from build123d import *

# Parameters (mm, degrees)
SKETCH_2_R              = 24
CUT_EXTRUDE_1_DEPTH     = 203.193286239
HOLE_WIZARD_M8_1_D      = 9
SKETCH_7_W              = 10
SKETCH_7_H              = 5
HOLE_WIZARD_M10_1_D     = 8.5
HOLE_WIZARD_M10_1_DEPTH = 24.5
HOLE_WIZARD_M10_1_TIP   = 2.553657631


with BuildPart() as part:
    # 草图1 → 旋转1 (revolve)
    with BuildSketch(Plane.XY, mode=Mode.PRIVATE) as revolve_1_sk:
        Polygon((0, 0), (87.5, 0), (87.5, 5), (111.25, 5), (111.25, 68), (80, 68), (80, 101), (42.5, 101), (42.5, 113), (27.5, 113), (27.5, 127), (0, 127), align=None)
    revolve(revolve_1_sk.sketch.rotate(Axis((0, 0, 0), (0, 1, 0)), 90), axis=Axis((0, 0, 0), (0, 1, 0)))

    # 草图2 → 切除-拉伸1 (cut, through all)
    with BuildSketch(Plane(origin=(0, 127, 0), x_dir=(1, 0, 0), z_dir=(0, 1, 0))):
        with Locations(Location((0, 0, 0), (0, 0, 270))):
            Circle(SKETCH_2_R)
    extrude(amount=-CUT_EXTRUDE_1_DEPTH, mode=Mode.SUBTRACT)

    # M8 间隙孔1 (through all)
    with Locations(Plane(origin=(0, 68, 0), x_dir=(1, 0, 0), z_dir=(0, 1, 0))):
        with Locations((0, 104), (73.539105243, 73.539105243), (104, 0), (73.539105243, -73.539105243), (0, -104), (-73.539105243, -73.539105243), (-104, 0), (-73.539105243, 73.539105243)):
            Hole(HOLE_WIZARD_M8_1_D / 2)

    # 草图7 → 切除-旋转1 (revolve, cut)
    with BuildSketch(Plane.XY, mode=Mode.PRIVATE) as cut_revolve_1_sk:
        with Locations((75, 91.5)):
            Rectangle(SKETCH_7_W, SKETCH_7_H)
    revolve(cut_revolve_1_sk.sketch.rotate(Axis((0, 0, 0), (0, 1, 0)), 90), axis=Axis((0, 0, 0), (0, 1, 0)), mode=Mode.SUBTRACT)

    # M10 螺纹孔1
    with Locations(Plane(origin=(0, 0, 0), x_dir=(-1, 0, 0), z_dir=(0, -1, 0))):
        with Locations((0, 67), (47.376154339, 47.376154339), (67, 0), (47.376154339, -47.376154339), (0, -67), (-47.376154339, -47.376154339), (-67, 0), (-47.376154339, 47.376154339)):
            Hole(HOLE_WIZARD_M10_1_D / 2, depth=HOLE_WIZARD_M10_1_DEPTH)
            with Locations((0, 0, -(HOLE_WIZARD_M10_1_DEPTH + HOLE_WIZARD_M10_1_TIP / 2))):  # 118° drill point
                Cone(0, HOLE_WIZARD_M10_1_D / 2, HOLE_WIZARD_M10_1_TIP, mode=Mode.SUBTRACT)


solid = part.part
Part model, mm, in its own coordinate system. A direction names the side the tool comes from. Round coordinates to 2 decimals unless told otherwise and drop trailing zeros. Order: outer loops, then holes, each group sorted by start corner. A loop starts at its lowest first (then second) coordinate and runs counter-clockwise, first axis right, second up. Notation, with made-up numbers: (-38.75, 51.5) -> (-14.75, 51.5) arc R20 ccw to (-14.75, 88.5) -> close; hole circle Ø7 at (38, 77). An arc over 180 degrees is marked (long way). Put each result on its own line as item: value.
Q1. Tool access for faces 4 (the face through (108.496, 36.059, -0.198)), 5 (the face through (71, 89, 0)), 6 (the face through (74, 68, -32)), 7 (the face through (-45.42, 12.42, 51.15)): list every direction of +Z, -Z, +X, -X, +Y, -Y with a clear straight run to the whole face (end or side of a thin tool).
From the geometry:
face 4: +Y, -Y
face 5: none
face 6: +Y
face 7: -Y
Q2. Pull direction X, two halves, no side cores. Call faces 1 (the face through (24.397, 120.098, -12.69)), 2 (the face through (7.21, 64.39, 22.89)), 3 (the face through (-1, 113, -28)): pulls with the +X half, pulls with the -X half, needs draft (parallel to the pull), parting line crosses it, or undercut.
From the geometry:
face 1: parting line crosses it
face 2: undercut
face 3: needs draft
Q3. Wall check: line 1 (Y direction, x = -32, z = 70.5); line 2 (X direction, y = 61, z = 76.5); line 3 (Y direction, x = -97.5, z = -33.5). Give the ranges that are in metal, low to high. Write a range as [from, to].
From the geometry:
line 1: y = [0, 89], [94, 101]
line 2: x = [-80.77, -76.93], [-70.15, 70.15], [76.93, 80.77]
line 3: y = [5, 68]
Q4. Band-saw the part on C-C (y = 33). State how many separate pieces and enclosed holes the cut face has, and give its area (3 significant figures).
From the geometry:
separate pieces: 1
enclosed holes: 9
area: 36,600 mm2
Q5. Band-saw the part on A-A (x = 104). Give the cut face in (y, z), and give its area (3 significant figures).
From the geometry:
outline: (5, -39.5) -> (68, -39.5) -> (68, -4.5) -> (5, -4.5) -> close; (5, 4.5) -> (68, 4.5) -> (68, 39.5) -> (5, 39.5) -> close
area: 4,410 mm2
Q6. Pin check, flat tips, straight feed: pin 1 Ø1 at (x, y) = (-23, 13.5) entering from -Z; pin 2 Ø7.5 at (x, z) = (-47.38, -47.38) entering from -Y; pin 3 Ø6 at (y, z) = (87, -63.5) entering from -X. Stop position of each tip, or through.
From the geometry:
pin 1: stops at z = -108.95
pin 2: stops at y = 24.8
pin 3: stops at x = -52.34
Q7. Band-saw the part on D-D (x = 55.5). Give the cut face in (y, z), and give its area (3 significant figures).
From the geometry:
outline: (0, -67.65) -> (5, -67.65) -> (5, -96.42) -> (68, -96.42) -> (68, -57.62) -> (89, -57.62) -> (89, -42.66) -> (94, -42.66) -> (94, -57.62) -> (101, -57.62) -> (101, 57.62) -> (94, 57.62) -> (94, 42.66) -> (89, 42.66) -> (89, 57.62) -> (68, 57.62) -> (68, 96.42) -> (5, 96.42) -> (5, 67.65) -> (0, 67.65) -> close
area: 16,500 mm2
